The figure shows three views and two pictorial views of one solid part (mm, origin at its lowest corner). Answer the questions. A direction names the side the tool comes from. Coordinates: 2 decimals unless noted, no trailing zeros. Order: outer loops, then holes, each group sorted by start corner. A loop starts at its lowest first (then second) coordinate and runs counter-clockwise, first axis right, second up. Notation, with made-up numbers: (34.5, 64) - (85.5, 64) arc R16 cw to (85.5, 79) - close; hole circle Ø2 at (-6.5, 23.25). An arc over 180 degrees is marked (long way). Answer as a JSON object with one key per item and string values. Group by question number.
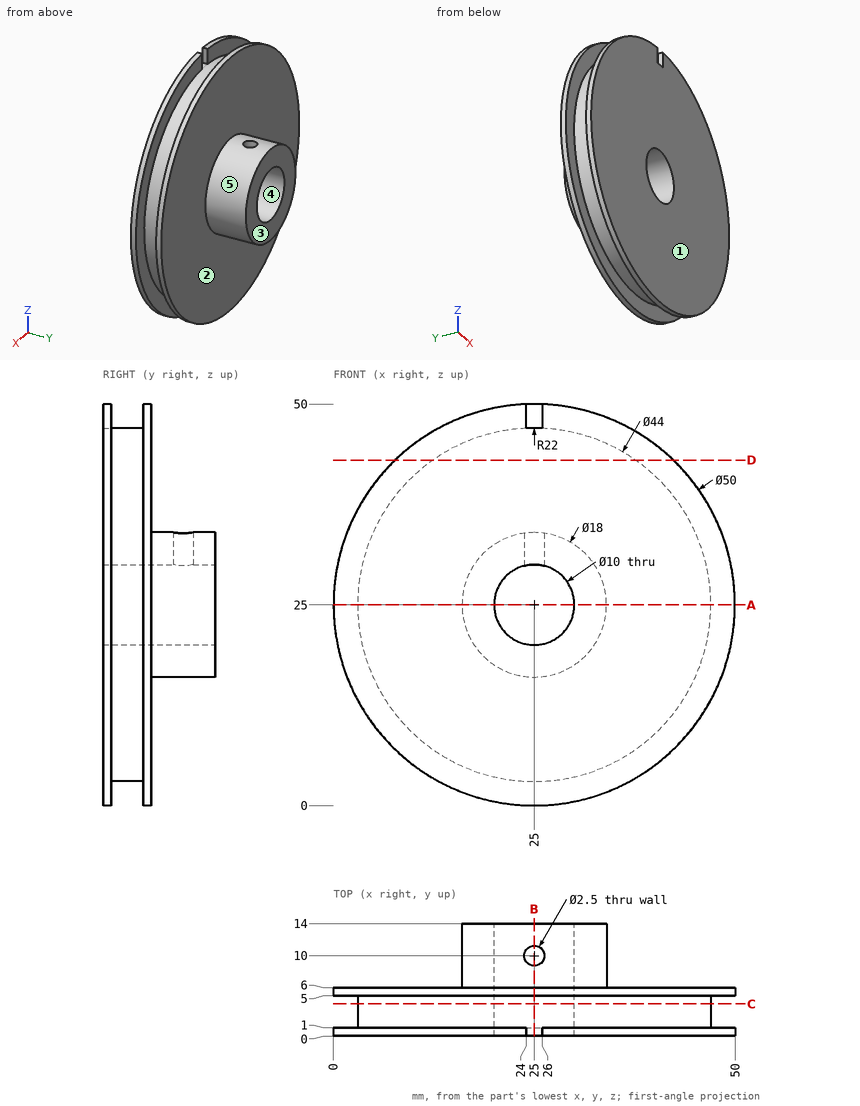
1. For the marked faces 1 and 2, determine the directions among +Z, -Z, +X, -X, +Y, -Y from which every point of the face is accessible in a straight line to the end or side of a thin tool.
2. For a pull along X with two mould halves and no side action, classify the marked faces 3, 4 and 5 as pulls with the +X half, pulls with the -X half, needs draft (parallel to the pull), parting line crosses it, or undercut.
3. A cutting plane is placed at C-C on y = 4. Write down the section's boundary in (x, z), and give its area (3 significant figures).
4. A cutting plane is placed at A-A on z = 25. Write down the section's boundary in (x, y).
5. Straight lines are drawn through the part: L1, parallel to Y at x = 25, z = 31.85; L2, parallel to Y at x = 7, z = 42; L3, parallel to X at y = 9, z = 25. For each, find the intervals that lie inside material, in ascending order.
6. Given pin 1 (5 mm diameter, centred on x = 27, y = 12, fed in from +Z); pin 2 (2 mm diameter, centred on x = 7.5, z = 43, fed in from -Y); pin 3 (0.8 mm diameter, centred on y = 0.5, z = 48, fed in from +X); pin 4 (12 mm diameter, centred on x = 43.5, z = 24.5, fed in from +Y), each flat-ended and moving along its own axis, determine where each tip first touches the part or whether it passes through.
7. A cutting plane is placed at B-B on x = 25. Write down the section's boundary in (y, z).
8. A cutting plane is placed at D-D on z = 43. Write down the section's boundary in (x, y).
Derived:
{
 "1": {"face 1": "+Z, -Z, +X, -X, -Y", "face 2": "+Y"},
 "2": {"face 3": "needs draft", "face 4": "undercut", "face 5": "parting line crosses it"},
 "3": {"outline": "circle Ø44 at (25, 25); hole circle Ø10 at (25, 25)", "area": "1,440 mm2"},
 "4": {"outline": "(0, 0) - (20, 0) - (20, 14) - (16, 14) - (16, 6) - (0, 6) - (0, 5) - (3, 5) - (3, 1) - (0, 1) - close; (30, 0) - (50, 0) - (50, 1) - (47, 1) - (47, 5) - (50, 5) - (50, 6) - (34, 6) - (34, 14) - (30, 14) - close"},
 "5": {"L1": "y = 0 to 8.75, 11.25 to 14", "L2": "y = 0 to 1, 5 to 6", "L3": "x = 16 to 20, 30 to 34"},
 "6": {"pin 1": "stops at z = 34", "pin 2": "stops at y = 0", "pin 3": "stops at x = 35.69", "pin 4": "stops at y = 6"},
 "7": {"outline": "(0, 0) - (1, 0) - (1, 3) - (5, 3) - (5, 0) - (6, 0) - (6, 16) - (14, 16) - (14, 20) - (0, 20) - close; (0, 30) - (8.75, 30) - (8.75, 34) - (6, 34) - (6, 50) - (5, 50) - (5, 47) - (0, 47) - close; (11.25, 30) - (14, 30) - (14, 34) - (11.25, 34) - close"},
 "8": {"outline": "(7.65, 0) - (42.35, 0) - (42.35, 1) - (37.65, 1) - (37.65, 5) - (42.35, 5) - (42.35, 6) - (7.65, 6) - (7.65, 5) - (12.35, 5) - (12.35, 1) - (7.65, 1) - close"}
}
